Read the model definition and answer for the solid it produces. Units are mm, in the model's axes. A direction names the side the tool comes from. Give positions to 0.01 mm unless a question says otherwise; leave off trailing zeros. Loops run counter-clockwise (first coordinate to the right, second up) from the corner with the lowest first, then second, coordinate; pieces in that order, holes last. Notation, with made-up numbers: (-9.5, 74) -> (26.5, 74) arc R23 cw to (26.5, 96) -> close; hole circle Ø10 at (40, 73). An arc over 180 degrees is marked (long way). One line per item, written item: value. Start each with the question number.
from build123d import *

# Parameters (mm, degrees)
BOSS_EXTRUDE1_DEPTH = 16
SKETCH2_R           = 5.5
CUT_EXTRUDE1_DEPTH  = 7
SKETCH3_R           = 3.5
CUT_EXTRUDE2_DEPTH  = 8
CHAMFER1_SIZE       = 1


with BuildPart() as part:
    # Sketch1 → Boss-Extrude1 (new body)
    with BuildSketch(Plane.XY):
        Polygon((0, 0), (0, 19), (26, 19), (26, 0), (22.5, 0), (22.5, 4), (3.5, 4), (3.5, 0), align=None)
    extrude(amount=BOSS_EXTRUDE1_DEPTH)

    # Sketch2 → Cut-Extrude1 (cut)
    with BuildSketch(Plane(origin=(0, 19, 0), x_dir=(1, 0, 0), z_dir=(0, 1, 0))):
        with Locations(Location((13, -8, 0), (0, 0, 270))):
            Circle(SKETCH2_R)
    extrude(amount=-CUT_EXTRUDE1_DEPTH, mode=Mode.SUBTRACT)

    # Sketch3 → Cut-Extrude2 (cut)
    with BuildSketch(Plane(origin=(0, 12, 0), x_dir=(1, 0, 0), z_dir=(0, 1, 0))):
        with Locations(Location((13, -8, 0), (0, 0, 270))):
            Circle(SKETCH3_R)
    extrude(amount=-CUT_EXTRUDE2_DEPTH, mode=Mode.SUBTRACT)

    # Chamfer1
    chamfer1_edges = [part.edges().sort_by_distance(p)[0] for p in [
        (0, 19, 8),
        (26, 19, 8),
    ]]
    chamfer(chamfer1_edges, length=CHAMFER1_SIZE)


solid = part.part
Item 1: A flat-ended cylindrical pin translates along its axis: pin 1 (2 mm diameter, centred on x = 9, z = 4, fed in from -Y). Find the tip coordinate at first contact, or state that the pin passes through.
Item 2: Section A-A, the plane x = 13 is taken. Determine the outline of the cut face in (y, z), plus the area to 3 significant figures.
Item 3: Consider L1, parallel to X at y = 15.25, z = 8; L2, parallel to X at y = 3.5, z = 2.5; L3, parallel to Y at x = 9.75, z = 11.75. Determine where each line is inside the solid, lowest interval first. Write a range as [from, to].
Item 4: For faces 4 (the cylindrical face through (10.89, 15.55, 13.08)), 5 (the flat face through (24, 0, 8)), 6 (the flat face through (3.5, 2, 8)), determine the directions among +Z, -Z, +X, -X, +Y, -Y from which every point of the face is accessible in a straight line to the end or side of a thin tool.
Item 5: Section B-B, the plane z = 8 is taken. Determine the outline of the cut face in (x, y), plus the area to 3 significant figures.
Item 6: Section D-D, the plane y = 17 is taken. Determine the outline of the cut face in (x, z), plus the area to 3 significant figures.
Item 7: Section C-C, the plane y = 1.75 is taken. Determine the outline of the cut face in (x, z), plus the area to 3 significant figures.
Item 8: Determine the mould class of faces 1 (the cylindrical face through (10.9, 8.1, 5.2)), 2 (the flat face through (13, 4, 4)), 3 (the flat face through (13, 12, 0)) for opening direction Z: pulls with the +Z half, pulls with the -Z half, needs draft (parallel to the pull), parting line crosses it, or undercut.
Computed values:
1. pin 1: y = 4
2. outline: (4, 0) -> (19, 0) -> (19, 2.5) -> (12, 2.5) -> (12, 4.5) -> (4, 4.5) -> close; (4, 11.5) -> (12, 11.5) -> (12, 13.5) -> (19, 13.5) -> (19, 16) -> (4, 16) -> close
2. area: 107 mm²
3. L1: [0, 7.5], [18.5, 26]
3. L2: [0, 3.5], [22.5, 26]
3. L3: [4, 12]
4. face 4: +Y
4. face 5: +Z, -Z, +X, -X, -Y
4. face 6: +Z, -Z, -Y
5. outline: (0, 0) -> (3.5, 0) -> (3.5, 4) -> (9.5, 4) -> (9.5, 12) -> (7.5, 12) -> (7.5, 19) -> (1, 19) -> (0, 18) -> close; (16.5, 4) -> (22.5, 4) -> (22.5, 0) -> (26, 0) -> (26, 18) -> (25, 19) -> (18.5, 19) -> (18.5, 12) -> (16.5, 12) -> close
5. area: 284 mm²
6. outline: (0, 0) -> (26, 0) -> (26, 16) -> (0, 16) -> close; hole circle Ø11 at (13, 8)
6. area: 321 mm²
7. outline: (0, 0) -> (3.5, 0) -> (3.5, 16) -> (0, 16) -> close; (22.5, 0) -> (26, 0) -> (26, 16) -> (22.5, 16) -> close
7. area: 112 mm²
8. face 1: undercut
8. face 2: needs draft
8. face 3: pulls with the -Z half
